from build123d import *

# Parameters (mm, degrees)
SKETCH_1_W          = 2266
SKETCH_1_H          = 880
EXTRUDE_1_DEPTH     = 40
SKETCH_2_W          = 1866
SKETCH_2_H          = 680
CUT_EXTRUDE_1_DEPTH = 1217.095802147
FILLET_1_R          = 100


with BuildPart() as part:
    # 草图1 → 凸台-拉伸1 (new body)
    with BuildSketch(Plane(origin=(0, 0, 0), x_dir=(1, 0, 0), z_dir=(0, 1, 0))):
        Rectangle(SKETCH_1_W, SKETCH_1_H)
    extrude(amount=EXTRUDE_1_DEPTH)

    # 草图2 → 切除-拉伸1 (cut, through all)
    with BuildSketch(Plane.XZ):
        Rectangle(SKETCH_2_W, SKETCH_2_H)
    extrude(amount=-CUT_EXTRUDE_1_DEPTH, mode=Mode.SUBTRACT)

    # 圆角1
    fillet_1_edges = [part.edges().sort_by_distance(p)[0] for p in [
        (933, 20, 340),
        (933, 20, -340),
        (-933, 20, -340),
        (-933, 20, 340),
    ]]
    fillet(fillet_1_edges, radius=FILLET_1_R)


solid = part.part
Verification items for the finished model (mm, model axes). A direction names the side the tool comes from. Coordinates: 2 decimals unless noted, no trailing zeros. Loops run counter-clockwise (first coordinate to the right, second up) from the corner with the lowest first, then second, coordinate; pieces in that order, holes last. Notation, with made-up numbers: (-14.5, -40) -> (44.5, -40) arc R18 ccw to (44.5, -7) -> close; hole circle Ø6 at (3.5, -29). An arc over 180 degrees is marked (long way). Write each question's results on one line, items separated by ' | '.
Item 1: Tool access check on faces 1 (the face through (-1133, 20, 6)), 2 (the face through (904.484, 20.28, -309.929)). Record the directions out of +Z, -Z, +X, -X, +Y, -Y that give a thin tool (end or side, any length) a straight path to the whole face; none if there is none.
Found:
face 1: +Z, -Z, -X, +Y, -Y | face 2: +Y, -Y
Item 2: Mould release check, pull along Z, two halves, no side actions. Record for faces 3 (the face through (-904.484, 20.28, 309.929)), 4 (the face through (-16, 20, -440)), 5 (the face through (-16, 0, 385)): +Z half, -Z half, draft (parallel to the pull), parting line (faces both ways), or undercut.
Found:
face 3: undercut | face 4: -Z half | face 5: draft
Item 3: Section check B-B, the plane z = -125. Enter the section's corners in (x, y), plus the area to 3 significant figures.
Found:
outline: (-1133, 0) -> (-933, 0) -> (-933, 40) -> (-1133, 40) -> close; (933, 0) -> (1133, 0) -> (1133, 40) -> (933, 40) -> close | area: 16,000 mm2
Item 4: Section check A-A, the plane x = 409. Enter the section's corners in (y, z).
Found:
outline: (0, -440) -> (40, -440) -> (40, -340) -> (0, -340) -> close; (0, 340) -> (40, 340) -> (40, 440) -> (0, 440) -> close
Item 5: Material ranges on L1, parallel to X at y = 8.5, z = -19.5; L2, parallel to Z at x = -671.5, y = 22.5; L3, parallel to X at y = 20, z = 295.5, recorded low to high.
Found:
L1: x = -1133 to -933, 933 to 1133 | L2: z = -440 to -340, 340 to 440 | L3: x = -1133 to -916.19, 916.19 to 1133
Item 6: Section check C-C, the plane y = 15.5. Enter the section's corners in (x, z), plus the area to 3 significant figures.
Found:
outline: (-1133, -440) -> (1133, -440) -> (1133, 440) -> (-1133, 440) -> close; hole (-933, -240) arc R100 ccw to (-833, -340) -> (833, -340) arc R100 ccw to (933, -240) -> (933, 240) arc R100 ccw to (833, 340) -> (-833, 340) arc R100 ccw to (-933, 240) -> close | area: 734,000 mm2
